Could you check a few things on this drawing? It's one solid part, dimensions in mm from its lowest x, y, z. Give positions to 0.01 mm unless a question says otherwise; leave off trailing zeros. Loops run counter-clockwise (first coordinate to the right, second up) from the corner with the lowest first, then second, coordinate; pieces in that order, holes last. Notation, with made-up numbers: (-1, 33.25) - (18, 33.25) arc R20 cw to (18, 39.25) - close; hole circle Ø9 at (7, 49). An arc over 180 degrees is marked (long way). Write item = value, one per line.
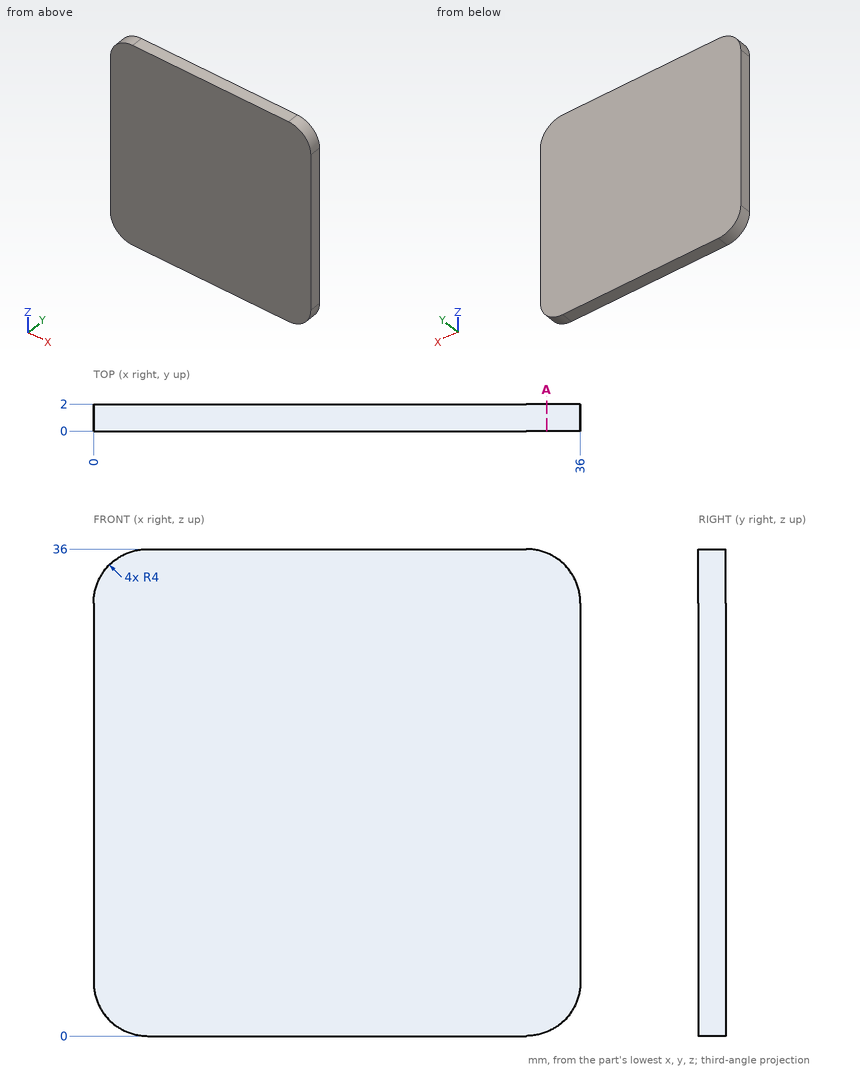
Q1. For pin 1 (6 mm diameter, centred on x = 27, z = 23.5, fed in from -Y), with a flat end and sliding along its axis, tell me the tip position at first contact or that it passes through.
Output:
pin_1 = 0
Q2. Imagine slicing it at A-A, the plane x = 33.5. Write out the boundary of the cut face in (y, z), then the cut area to 3 significant figures.
Output:
outline = (0, 0.29) - (2, 0.29) - (2, 35.71) - (0, 35.71) - close
area = 70.8 mm2
Q3. I need wall thicknesses on L1, parallel to Z at x = 2, y = 0.8; L2, parallel to Z at x = 33.5, y = 1.2; L3, parallel to X at y = 0.15, z = 33. Which ranges of each line are inside material? Lowest first, please.
Output:
L1 = 0.54 to 35.46
L2 = 0.29 to 35.71
L3 = 0.13 to 35.87
